```python
from build123d import *

# Parameters (mm, degrees)
EXTRUDE_378_DEPTH      = 5.3
SKETCH_4_W             = 0.6
SKETCH_4_H             = 11.005553499
CHAMFER_2060_SIZE      = 1
FILLET_2105_R          = 0.4
PATTERN_LINEAR_1_COUNT = 9
PATTERN_LINEAR_1_PITCH = 1.25


with BuildPart() as part:
    # 草图1 → Extrude 378 (new body)
    with BuildSketch(Plane(origin=(0, 0, 0), x_dir=(0, 0, -1), z_dir=(1, 0, 0))):
        Polygon((6.5, 3.75277675), (6.5, -3.75277675), (0, -7.505553499), (-6.5, -3.75277675), (-6.5, 3.75277675), (0, 7.505553499), align=None)
    extrude(amount=EXTRUDE_378_DEPTH)

    # 草图2 → 凸台-旋转1 (revolve)
    with BuildSketch(Plane.XY, mode=Mode.PRIVATE) as revolve_1_sk:
        Polygon((0, 0), (35.3, 0), (35.3, 2.9175), (35.3, 4), (7.791693541, 4), (0, 4), align=None)
    revolve(revolve_1_sk.sketch.rotate(Axis((0, 0, 0), (1, 0, 0)), 90), axis=Axis((0, 0, 0), (1, 0, 0)))

    # 草图3 → 切除-旋转1 (revolve, cut)
    with BuildSketch(Plane.XY):
        Polygon((0, 6.5), (3.46730793, 12.505553499), (3.46730793, 17.505553499), (-10, 17.505553499), (-10, 6.5), align=None)
    revolve(axis=Axis((0, 0, 0), (1, 0, 0)), mode=Mode.SUBTRACT)

    # 草图5 → 切除-旋转2 (revolve, cut)
    with BuildSketch(Plane.XY):
        Polygon((5.3, 6.5), (1.83269207, 12.505553499), (1.83269207, 17.505553499), (11.83269207, 17.505553499), (11.83269207, 6.5), align=None)
    revolve(axis=Axis((0, 0, 0), (1, 0, 0)), mode=Mode.SUBTRACT)

    # 草图4 → 切除-旋转3 (revolve, cut)
    with BuildSketch(Plane.XY, mode=Mode.PRIVATE) as cut_revolve_3_sk:
        with Locations((5, 12.00277675)):
            Rectangle(SKETCH_4_W, SKETCH_4_H)
    revolve(cut_revolve_3_sk.sketch.rotate(Axis((0, 0, 0), (1, 0, 0)), 270), axis=Axis((0, 0, 0), (1, 0, 0)), mode=Mode.SUBTRACT)

    # Chamfer 2060
    chamfer_2060_edges = [part.edges().sort_by_distance(p)[0] for p in [
        (35.3, 0, -4),
    ]]
    chamfer(chamfer_2060_edges, length=CHAMFER_2060_SIZE)

    # Fillet 2105
    fillet_2105_edges = [part.edges().sort_by_distance(p)[0] for p in [
        (5.3, 0, -4),
    ]]
    fillet(fillet_2105_edges, radius=FILLET_2105_R)

    # 草图6 → 切除-旋转4 (revolve, cut)
    with BuildSketch(Plane.XY):
        Polygon((25.3, -2.9175), (24.675018334, -4), (24.675018334, -5), (25.924981666, -5), (25.924981666, -4), align=None)
    cut_revolve_4 = revolve(axis=Axis((-3.175, 0, 0), (1, 0, 0)), mode=Mode.SUBTRACT)

    # 阵列(线性)1: 切除-旋转4 ×9
    with Locations(*[(i * PATTERN_LINEAR_1_PITCH, 0, 0) for i in range(1, PATTERN_LINEAR_1_COUNT)]):
        add(cut_revolve_4, mode=Mode.SUBTRACT)


solid = part.part
```
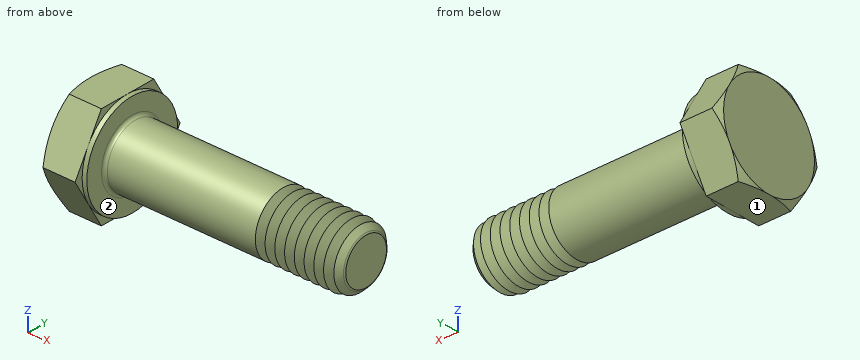
CAD build for the part. Positions are in the model's coordinates, mm. Face numbers are marked on the shaded views. A direction names the side the tool comes from. Round coordinates to 2 decimals unless told otherwise and drop trailing zeros. Order: outer loops, then holes, each group sorted by start corner. A loop starts at its lowest first (then second) coordinate and runs counter-clockwise, first axis right, second up.
Q1. Slice it at A-A (x = 17.5). Write the cut outline in (y, z).
Q2. Wall check: L1, parallel to X at y = 0.75, z = 4.25; L2, parallel to Z at x = 15, y = 0.25; L3, parallel to Z at x = 7.5, y = -2. Give the ranges that are in metal, low to high.
Q3. Drop flat-ended pins along their axis: pin 1 (1.6 mm diameter, centred on y = -2, z = 5.5, fed in from +X); pin 2 (1.5 mm diameter, centred on x = 18.5, z = 2.5, fed in from -Y); pin 3 (8 mm diameter, centred on x = 11.5, y = 1.5, fed in from -Z). Give the stop position or say it passes through.
Q4. Which spindle directions (+Z, -Z, +X, -X, +Y, -Y) get a long thin tool onto all of the face, cutting with end or side? Do the marked faces 1 and 2. Say none if no direction does.
Results below:
1. outline: circle Ø8 at (0, 0)
2. L1: x = 0 to 5.31
2. L2: z = -3.99 to 3.99
2. L3: z = -3.46 to 3.46
3. pin 1: stops at x = 5.3
3. pin 2: stops at y = -3.6
3. pin 3: stops at z = -4
4. face 1: -Z, +X, -X, +Y, -Y
4. face 2: +X
